Source: CAD feature listing. Evaluate the final solid. Frame: model axes, mm. Face numbers are marked on the shaded views. Give positions to 0.01 mm unless a question says otherwise; leave off trailing zeros. Order: outer loops, then holes, each group sorted by start corner. A loop starts at its lowest first (then second) coordinate and runs counter-clockwise, first axis right, second up. Notation, with made-up numbers: (50, -11) - (107, -11) arc R24 cw to (107, 0) - close; hole circle Ø1 at (-9.75, 59.25). An arc over 180 degrees is marked (long way). One line per item, written item: value. Start each with the question number.
from build123d import *

# Parameters (mm, degrees)
SKETCH1_R           = 26.5
BOSS_EXTRUDE1_DEPTH = 200
SKETCH2_R           = 23.5
CUT_EXTRUDE1_DEPTH  = 200
CHAMFER1_SIZE       = 0.5
SKETCH4_W           = 1.5
SKETCH4_H           = 53
CUT_EXTRUDE2_DEPTH  = 180
CIRPATTERN1_COUNT   = 2
CIRPATTERN1_ANGLE   = 90
CUT_EXTRUDE3_DEPTH  = 180
CIRPATTERN2_COUNT   = 2
CIRPATTERN2_ANGLE   = 90


with BuildPart() as part:
    # Sketch1 → Boss-Extrude1 (new body)
    with BuildSketch(Plane.XY):
        Circle(SKETCH1_R)
    extrude(amount=BOSS_EXTRUDE1_DEPTH)

    # Sketch2 → Cut-Extrude1 (cut)
    with BuildSketch(Plane(origin=(0, 0, 0), x_dir=(-1, 0, 0), z_dir=(0, 0, -1))):
        Circle(SKETCH2_R)
    extrude(amount=-CUT_EXTRUDE1_DEPTH, mode=Mode.SUBTRACT)

    # Chamfer1
    chamfer1_edges = [part.edges().sort_by_distance(p)[0] for p in [
        (-26.5, 0, 0),
        (-26.5, 0, 200),
        (23.5, 0, 200),
        (23.5, 0, 0),
    ]]
    chamfer(chamfer1_edges, length=CHAMFER1_SIZE)

    # Sketch4 → Cut-Extrude2 (cut)
    with BuildSketch(Plane.XY.offset(200)):
        Rectangle(SKETCH4_W, SKETCH4_H)
    cut_extrude2 = extrude(amount=-CUT_EXTRUDE2_DEPTH, mode=Mode.SUBTRACT)

    # CirPattern1: Cut-Extrude2 ×2 about axis
    cirpattern1_axis = Axis((0, 0, 199.5), (0, 0, -1))
    for i in range(1, CIRPATTERN1_COUNT):
        add(cut_extrude2.rotate(cirpattern1_axis, i * CIRPATTERN1_ANGLE / (CIRPATTERN1_COUNT - 1)), mode=Mode.SUBTRACT)

    # Sketch5 → Cut-Extrude3 (cut)
    with BuildSketch(Plane(origin=(0, 0, 0), x_dir=(-1, 0, 0), z_dir=(0, 0, -1))):
        Polygon((-21.214455758, 20.159230222), (21.211951113, -22.267176649), (22.269893967, -21.209233795), (-20.156512904, 21.217173076), align=None)
    cut_extrude3 = extrude(amount=-CUT_EXTRUDE3_DEPTH, mode=Mode.SUBTRACT)

    # CirPattern2: Cut-Extrude3 ×2 about axis
    cirpattern2_axis = Axis((0, 0, 199.5), (0, 0, -1))
    for i in range(1, CIRPATTERN2_COUNT):
        add(cut_extrude3.rotate(cirpattern2_axis, i * CIRPATTERN2_ANGLE / (CIRPATTERN2_COUNT - 1)), mode=Mode.SUBTRACT)


solid = part.part
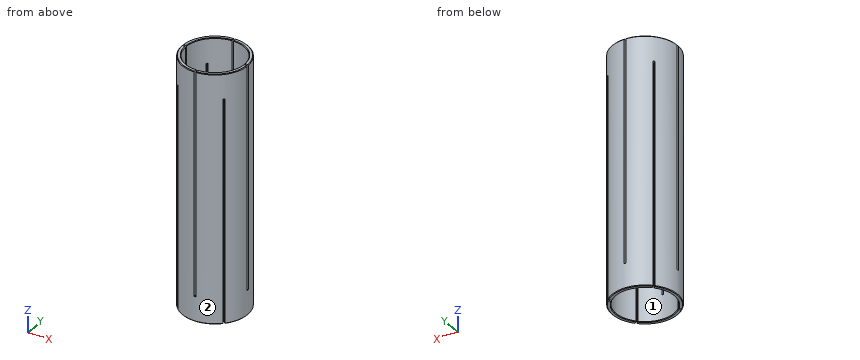
1. Draft query along X for the marked faces 1 and 2. Return one class per face: pulls with the +X half, pulls with the -X half, needs draft (parallel to the pull), parting line crosses it, or undercut.
2. Contact query for flat-ended pins moving along their axis: pin 1 Ø6 at (x, z) = (-17.5, 30) entering from -Y; pin 2 Ø6 at (x, z) = (-8.5, 90.5) entering from -Y; pin 3 Ø0.9 at (y, z) = (-24, 101) entering from +X; pin 4 Ø12 at (x, y) = (-20, 20.5) entering from +Z. Output: stop coordinate, or through.
3. Ray query, L1, parallel to Y at x = -18, z = 132; L2, parallel to X at y = 18.5, z = 152; L3, parallel to Y at x = -20, z = 162.5. Return the intervals inside material, ascending.
4. Section A-A on z = 182.5. Return the cut outline in (x, y).
5. Section B-B on z = 66. Count the separate pieces of the cut face and the enclosed holes in it, then the cut area to 3 significant figures.
Data:
1. face 1: undercut
1. face 2: parting line crosses it
2. pin 1: stops at y = -22.18
2. pin 2: stops at y = -25.92
2. pin 3: stops at x = 12.15
2. pin 4: stops at z = 200
3. L1: y = -19.45 to -19.06, -16.94 to -15.11, 15.11 to 16.94, 19.06 to 19.45
3. L2: x = -17.44 to -14.49, 14.49 to 17.44
3. L3: y = -17.39 to -12.34, 12.34 to 17.39
4. outline: (-26.49, -0.75) arc R26.5 ccw to (-0.75, -26.49) - (-0.75, -23.49) arc R23.5 cw to (-23.49, -0.75) - close; (-26.49, 0.75) - (-23.49, 0.75) arc R23.5 cw to (-0.75, 23.49) - (-0.75, 26.49) arc R26.5 ccw to start; (0.75, -26.49) arc R26.5 ccw to (26.49, -0.75) - (23.49, -0.75) arc R23.5 cw to (0.75, -23.49) - close; (0.75, 23.49) arc R23.5 cw to (23.49, 0.75) - (26.49, 0.75) arc R26.5 ccw to (0.75, 26.49) - close
5. separate pieces: 8
5. enclosed holes: 0
5. area: 435 mm2
